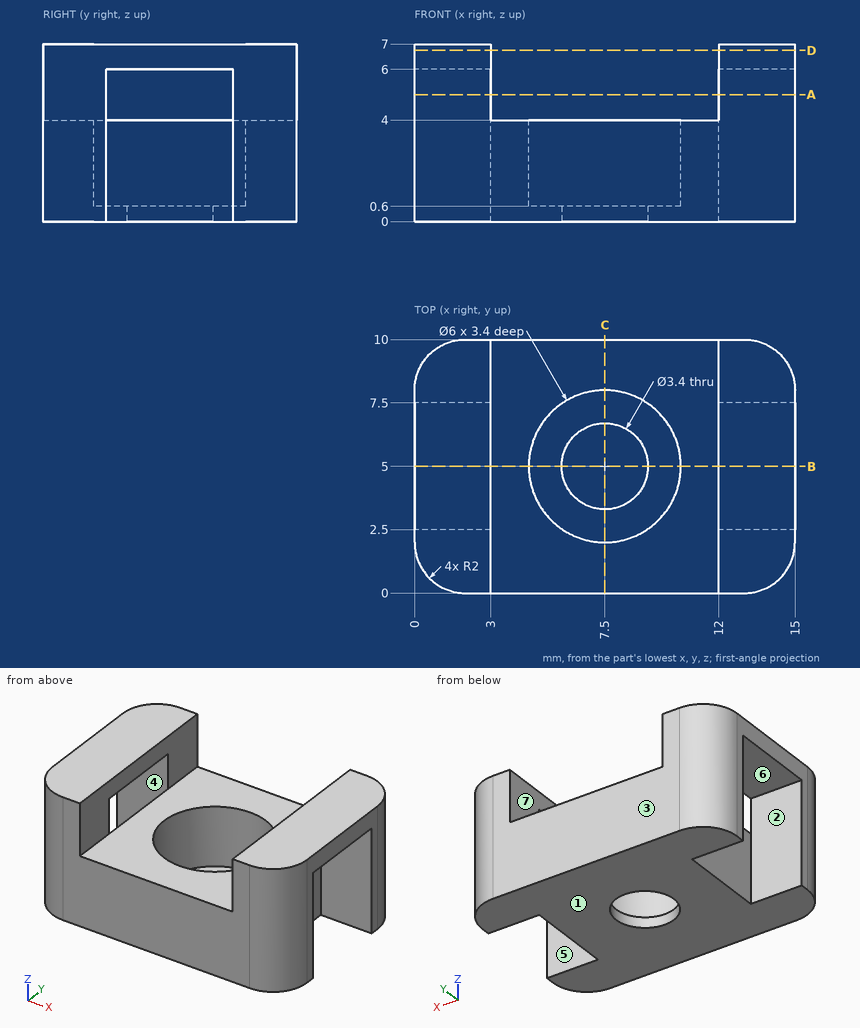
Part print with two shaded views. Sizes in mm from the minimum x, y, z corner. A direction names the side the tool comes from. Round coordinates to 2 decimals unless told otherwise and drop trailing zeros. Order: outer loops, then holes, each group sorted by start corner. A loop starts at its lowest first (then second) coordinate and runs counter-clockwise, first axis right, second up. Notation, with made-up numbers: (-16.5, 48) -> (8.5, 48) arc R16 cw to (8.5, 75) -> close; hole circle Ø9 at (-25, -31). An arc over 180 degrees is marked (long way). One line per question, with ' | ' between items.
Q1. Which spindle directions (+Z, -Z, +X, -X, +Y, -Y) get a long thin tool onto all of the face, cutting with end or side? Do the marked faces 4, 5, 6 and 7. Say none if no direction does.
Completed:
face 4: -Z, -X | face 5: -Z, +X | face 6: -Z, +X, -X | face 7: +Z, +Y, -Y
Q2. Probe probe 1 along Y at (x, z) = (7.5, 1.55); probe 2 along Y at (x, z) = (7.5, 0.3); probe 3 along Z at (x, y) = (9.5, 1.25). List the from-to ranges inside material, lowest first.
Completed:
probe 1: y = 0 to 2, 8 to 10 | probe 2: y = 0 to 3.3, 6.7 to 10 | probe 3: z = 0 to 4
Q3. Slice it at D-D (z = 6.75). Write the cut outline in (x, y), then the cut area to 3 significant figures.
Completed:
outline: (0, 2) arc R2 ccw to (2, 0) -> (3, 0) -> (3, 10) -> (2, 10) arc R2 ccw to (0, 8) -> close; (12, 0) -> (13, 0) arc R2 ccw to (15, 2) -> (15, 8) arc R2 ccw to (13, 10) -> (12, 10) -> close | area: 56.6 mm^2
Q4. Drop flat-ended pins along their axis: pin 1 (0.9 mm diameter, centred on x = 2, y = 5, fed in from -Z); pin 2 (0.9 mm diameter, centred on x = 2, z = 3.5, fed in from -Y); pin 3 (0.9 mm diameter, centred on x = 1, z = 2.5, fed in from +Y); pin 4 (1.2 mm diameter, centred on y = 4, z = 1.5, fed in from -X). Give the stop position or say it passes through.
Completed:
pin 1: stops at z = 6 | pin 2: stops at y = 0 | pin 3: stops at y = 9.92 | pin 4: stops at x = 3
Q5. Slice it at B-B (y = 5). Write the cut outline in (x, z), then the cut area to 3 significant figures.
Completed:
outline: (0, 6) -> (3, 6) -> (3, 7) -> (0, 7) -> close; (3, 0) -> (5.8, 0) -> (5.8, 0.6) -> (4.5, 0.6) -> (4.5, 4) -> (3, 4) -> close; (9.2, 0) -> (12, 0) -> (12, 4) -> (10.5, 4) -> (10.5, 0.6) -> (9.2, 0.6) -> close; (12, 6) -> (15, 6) -> (15, 7) -> (12, 7) -> close | area: 19.6 mm^2
Q6. Slice it at A-A (z = 5). Write the cut outline in (x, y).
Completed:
outline: (0, 2) arc R2 ccw to (2, 0) -> (3, 0) -> (3, 2.5) -> (0, 2.5) -> close; (0, 7.5) -> (3, 7.5) -> (3, 10) -> (2, 10) arc R2 ccw to (0, 8) -> close; (12, 0) -> (13, 0) arc R2 ccw to (15, 2) -> (15, 2.5) -> (12, 2.5) -> close; (12, 7.5) -> (15, 7.5) -> (15, 8) arc R2 ccw to (13, 10) -> (12, 10) -> close
Q7. Two-plate mould, pull along Y, no slides. Class the marked faces 1, 2 and 3: released by +Y, released by -Y, zero draft, split by the parting line, or undercut.
Completed:
face 1: zero draft | face 2: undercut | face 3: released by +Y
Q8. Slice it at C-C (x = 7.5). Write the cut outline in (y, z), then the cut area to 3 significant figures.
Completed:
outline: (0, 0) -> (3.3, 0) -> (3.3, 0.6) -> (2, 0.6) -> (2, 4) -> (0, 4) -> close; (6.7, 0) -> (10, 0) -> (10, 4) -> (8, 4) -> (8, 0.6) -> (6.7, 0.6) -> close | area: 17.6 mm^2
